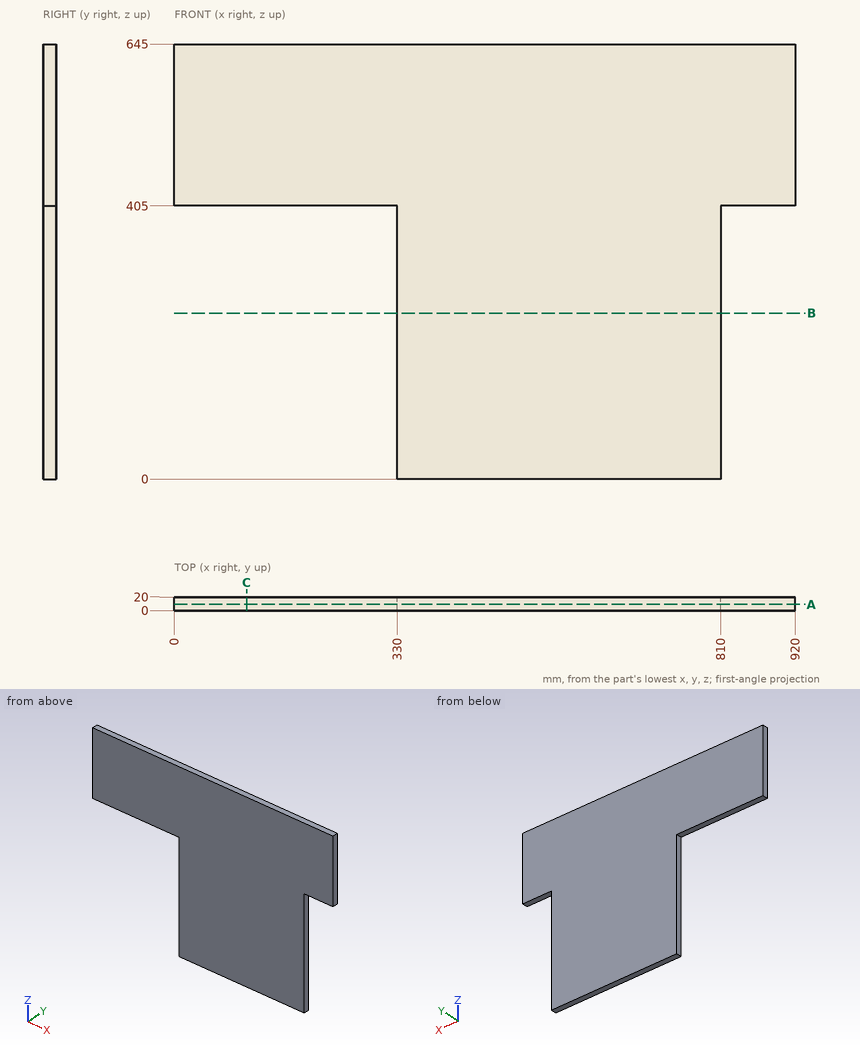
Geometry check sheet. Reference: drawing and pictorial views, mm from the part's lowest x, y, z. Coordinates: 2 decimals unless noted, no trailing zeros. Write each loop counter-clockwise with the first axis right and the second up, starting at its lowest first coordinate (ties: lowest second). Pieces come first, ordered by that corner, then holes. Notation, with made-up numbers: (-15.5, 30.5) -> (5.5, 30.5) arc R20 cw to (5.5, 46.5) -> close; hole circle Ø5 at (17.5, 69.5). An arc over 180 degrees is marked (long way). One line per question, with ' | ' between items.
1. Thickness scan on probe 1 along Z at (x, y) = (283, 7); probe 2 along X at (y, z) = (6.25, 161.5). Record the ranges inside material, lowest first. Write a range as from..to.
Answers:
probe 1: z = 405..645 | probe 2: x = 330..810
2. Depth check by flat-ended pin: pin 1 Ø6 at (x, y) = (217.5, 7) entering from -Z; pin 2 Ø1.5 at (y, z) = (12.5, 106) entering from -X; pin 3 Ø10 at (y, z) = (14, 109) entering from +X. Enter the tip coordinate at first touch or a pass-through.
Answers:
pin 1: stops at z = 405 | pin 2: stops at x = 330 | pin 3: stops at x = 810
3. Cross-section at B-B on z = 246. Record the cut outline in (x, y), and give its area (3 significant figures).
Answers:
outline: (330, 0) -> (810, 0) -> (810, 20) -> (330, 20) -> close | area: 9,600 mm²
4. Cross-section at C-C on x = 107. Record the cut outline in (y, z).
Answers:
outline: (0, 405) -> (20, 405) -> (20, 645) -> (0, 645) -> close
5. Cross-section at A-A on y = 9. Record the cut outline in (x, z).
Answers:
outline: (0, 405) -> (330, 405) -> (330, 0) -> (810, 0) -> (810, 405) -> (920, 405) -> (920, 645) -> (0, 645) -> close
